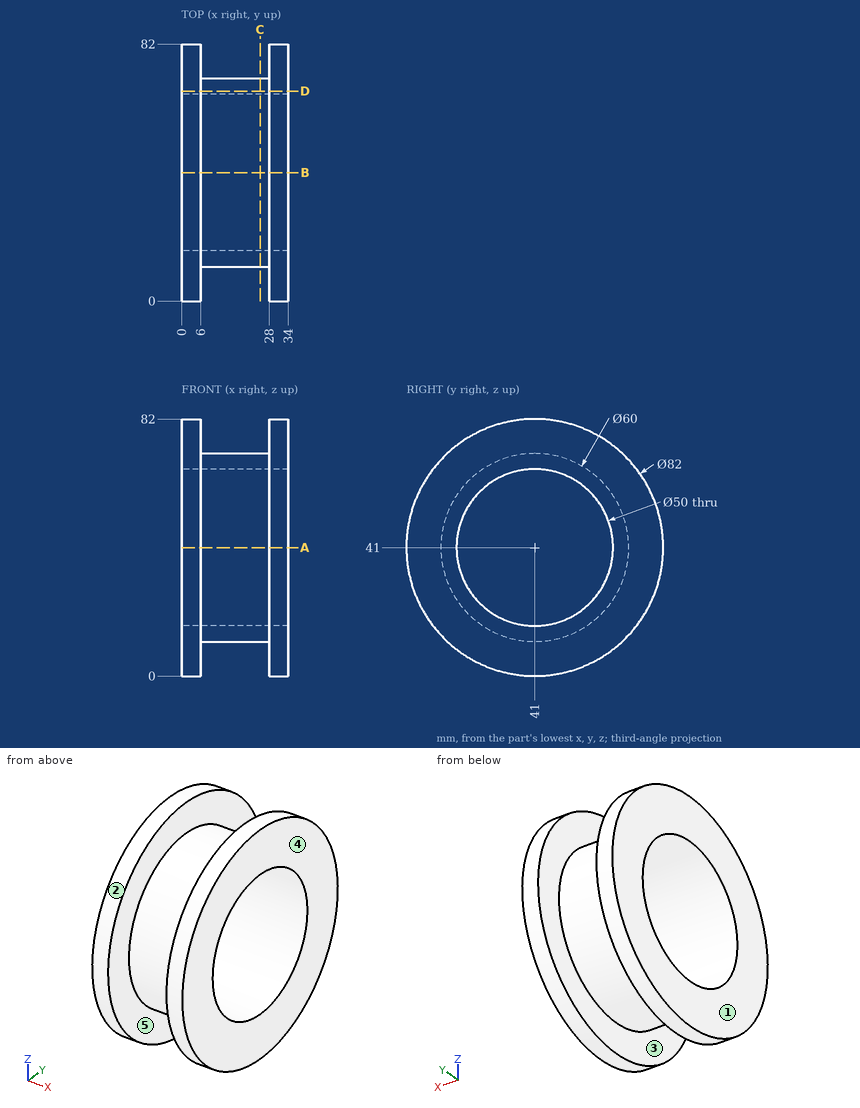
Input: dimensioned drawing with shaded views. Units: mm. Origin: part minimum x, y, z. A direction names the side the tool comes from. Round coordinates to 2 decimals unless told otherwise and drop trailing zeros. Loops run counter-clockwise (first coordinate to the right, second up) from the corner with the lowest first, then second, coordinate; pieces in that order, holes last. Notation, with made-up numbers: (-14, -33) -> (23, -33) arc R22 ccw to (23, -7) -> close; hole circle Ø8 at (19, -16.5). An arc over 180 degrees is marked (long way). Answer as a JSON object with one key per item and string values. Group by question number.
1) Section query C-C on x = 25. Output: boundary loops of the cut face in (y, z), plus the area to 3 significant figures.
2) Pin query (flat end, axial travel): pin 1 (1.5 mm diameter, centred on x = 27.5, y = 45.5, fed in from -Z); pin 2 (24.5 mm diameter, centred on y = 58.5, z = 33, fed in from +X); pin 3 (5 mm diameter, centred on x = 4.5, z = 40, fed in from +Y); pin 4 (6 mm diameter, centred on x = 14.5, y = 69.5, fed in from -Z). Return the tip coordinate at first contact, or that it passes through.
3) Section query A-A on z = 41. Output: boundary loops of the cut face in (x, y).
4) Section query D-D on y = 67. Output: boundary loops of the cut face in (x, z).
5) Reachability of the marked faces 4 and 5 from +Z, -Z, +X, -X, +Y, -Y: full face, straight path, thin tool, end or side. Return the list, or none.
6) Ray query, L1, parallel to Y at x = 17, z = 41; L2, parallel to X at y = 36, z = 77. Return the intervals inside material, ascending.
7) Draft query along X for the marked faces 1, 2 and 3. Return one class per face: +X half, -X half, draft (parallel to the pull), parting line (faces both ways), or undercut.
Reply:
{
 "1": {"outline": "circle Ø60 at (41, 41); hole circle Ø50 at (41, 41)", "area": "864 mm2"},
 "2": {"pin 1": "stops at z = 0.19", "pin 2": "stops at x = 34", "pin 3": "stops at y = 82", "pin 4": "stops at z = 25.2"},
 "3": {"outline": "(0, 0) -> (6, 0) -> (6, 11) -> (28, 11) -> (28, 0) -> (34, 0) -> (34, 16) -> (0, 16) -> close; (0, 66) -> (34, 66) -> (34, 82) -> (28, 82) -> (28, 71) -> (6, 71) -> (6, 82) -> (0, 82) -> close"},
 "4": {"outline": "(0, 9.3) -> (6, 9.3) -> (6, 26.03) -> (28, 26.03) -> (28, 9.3) -> (34, 9.3) -> (34, 72.7) -> (28, 72.7) -> (28, 55.97) -> (6, 55.97) -> (6, 72.7) -> (0, 72.7) -> close"},
 "5": {"face 4": "+Z, -Z, +X, +Y, -Y", "face 5": "none"},
 "6": {"L1": "y = 11 to 16, 66 to 71", "L2": "x = 0 to 6, 28 to 34"},
 "7": {"face 1": "-X half", "face 2": "draft", "face 3": "undercut"}
}
